from build123d import *

# Parameters (mm, degrees)
SLOTTED_BRACKET_BODY_DEPTH = 6
LUG_A_SKETCH_R             = 6.5
MOUNTING_LUG_A_13_DEPTH    = 6
LUG_B_SKETCH_R             = 6.5
MOUNTING_LUG_B_13_DEPTH    = 6


with BuildPart() as part:
    # Bracket Profile Sketch → Slotted Bracket Body (new body)
    with BuildSketch(Plane.XY):
        with BuildLine():
            Line((-35.440613027, 25), (-35.440613027, 0))
            Line((-35.440613027, 0), (34.559386973, 0))
            Line((34.559386973, 0), (34.559386973, 6))
            Line((34.559386973, 6), (14.559386973, 6))
            ThreePointArc((14.559386973, 6), (8.059386973, 12.5), (14.559386973, 19))
            ThreePointArc((14.559386973, 19), (14.640630626, 18.999492247), (14.721861587, 18.997969067))
            Line((14.721861587, 18.997969067), (34.559386973, 18.75))
            Line((34.559386973, 18.75), (34.559386973, 25))
            Line((34.559386973, 25), (-35.440613027, 25))
        make_face()
    extrude(amount=SLOTTED_BRACKET_BODY_DEPTH)

    # Lug A Sketch → Mounting Lug A Ø13 (add)
    with BuildSketch(Plane.ZY.offset(35.440613027)):
        with BuildLine():
            Line((-18, 0), (6, 0))
            Line((6, 0), (6, 25))
            Line((6, 25), (-18, 25))
            ThreePointArc((-18, 25), (-30.5, 12.5), (-18, 0))
        make_face()
        with Locations((-18, 12.5)):
            Circle(LUG_A_SKETCH_R, mode=Mode.SUBTRACT)
    extrude(amount=-MOUNTING_LUG_A_13_DEPTH)

    # Lug B Sketch → Mounting Lug B Ø13 (add)
    with BuildSketch(Plane.XZ):
        with BuildLine():
            Line((-35.440613027, 18), (-35.440613027, 0))
            Line((-35.440613027, 0), (-10.440613027, 0))
            Line((-10.440613027, 0), (-10.440613027, 18))
            ThreePointArc((-10.440613027, 18), (-22.940613027, 30.5), (-35.440613027, 18))
        make_face()
        with Locations(Location((-22.940613027, 18, 0), (0, 0, 270))):
            Circle(LUG_B_SKETCH_R, mode=Mode.SUBTRACT)
    extrude(amount=-MOUNTING_LUG_B_13_DEPTH)


solid = part.part
Read the model definition and answer for the solid it produces. Units are mm, in the model's axes. A direction names the side the tool comes from. Round coordinates to 2 decimals unless told otherwise and drop trailing zeros. Write each loop counter-clockwise with the first axis right and the second up, starting at its lowest first coordinate (ties: lowest second). Pieces come first, ordered by that corner, then holes.
Q1. Flat-ended cylindrical pins translate along their axes: P1, Ø12.5, axis at x = 16, y = 10.5, coming from the +Z side; P2, Ø7.5, axis at x = -24.5, z = 20, coming from the +Y side; P3, Ø6.5, axis at y = 3.5, z = 11.5, coming from the +X side; P4, Ø7.5, axis at x = -9.5, y = 9.5, coming from the -Z side. Find the tip coordinate at first contact, or state that the pin passes through.
Values:
P1: stops at z = 6
P2: passes through
P3: stops at x = -10.44
P4: stops at z = 0
Q2. Straight lines are drawn through the part: line 1 (Y direction, x = -31, z = -18); line 2 (X direction, y = 12.75, z = 3.5); line 3 (X direction, y = 18.75, z = -23). For each, find the intervals that lie inside material, in ascending order.
Values:
line 1: y = 0 to 6, 19 to 25
line 2: x = -35.44 to 8.06
line 3: x = -35.44 to -29.44
Q3. The mould has two halves that part along Z. Classify faces 1 (the face through (-32.483, 12.786, -24.494)), 2 (the face through (-8, 25, 1)), 3 (the face through (-22.666, 2.958, 30.497)): released by +Z, released by -Z, zero draft, split by the parting line, or undercut.
Values:
face 1: undercut
face 2: zero draft
face 3: released by +Z
Q4. Find section A-A on y = 12.5. Determine the outline of the cut face in (x, z).
Values:
outline: (-35.44, -30.5) - (-29.44, -30.5) - (-29.44, -24.5) - (-35.44, -24.5) - close; (-35.44, -11.5) - (-29.44, -11.5) - (-29.44, 0) - (8.06, 0) - (8.06, 6) - (-35.44, 6) - close
Q5. Find section C-C on y = 4.75. Determine the outline of the cut face in (x, z).
Values:
outline: (-35.44, -27.81) - (-29.44, -27.81) - (-29.44, 0) - (34.56, 0) - (34.56, 6) - (-10.44, 6) - (-10.44, 18) arc R12.5 ccw to (-35.44, 18) - close; hole circle Ø13 at (-22.94, 18)
Q6. Find section B-B on z = 12.5. Determine the outline of the cut face in (x, y), and give its area (3 significant figures).
Values:
outline: (-35.44, 0) - (-26.4, 0) - (-26.4, 6) - (-35.44, 6) - close; (-19.48, 0) - (-10.44, 0) - (-10.44, 6) - (-19.48, 6) - close
area: 108 mm2
Q7. Find section D-D on x = -20.5. Determine the outline of the cut face in (y, z), and give its area (3 significant figures).
Values:
outline: (0, 0) - (25, 0) - (25, 6) - (6, 6) - (6, 11.98) - (0, 11.98) - close; (0, 24.02) - (6, 24.02) - (6, 30.26) - (0, 30.26) - close
area: 223 mm2
Q8. A tool of negligible diameter and unlimited length cuts with its end or side. For faces 4 (the face through (-10.441, 3, 12)), 5 (the face through (-29.441, 13, -9)), 6 (the face through (25, 6, 3)), 7 (the face through (-23, 6, 10)), from which of +Z, -Z, +X, -X, +Y, -Y can it reach the whole face along a straight path? Write none if from no direction.
Values:
face 4: +Z, +X, +Y, -Y
face 5: -Z, +X, +Y, -Y
face 6: +Z, -Z, +X
face 7: +Z, +X, -X, +Y
